from build123d import *

# Parameters (mm, degrees)
SKETCH2_W            = 12
SKETCH2_H            = 35.5
BOSS_EXTRUDE1_DEPTH  = 7.5
LPATTERN1_COUNT      = 2
LPATTERN1_PITCH      = 587
BOSS_EXTRUDE2_DEPTH  = 15
M5_CLEARANCE_HOLE1_D = 5.5
M5_CLEARANCE_HOLE2_D = 5.5


with BuildPart() as part:
    # Sketch1 → Revolve1 (revolve)
    with BuildSketch(Plane.XY):
        Polygon((0, 0), (0, 10.5), (29, 10.5), (29, 9.5), (39, 9.5), (39, 10.5), (75, 10.5), (75, 10), (625, 10), (625, 10.5), (661, 10.5), (661, 9.5), (671, 9.5), (671, 10.5), (700, 10.5), (700, 0), align=None)
    revolve(axis=Axis((700, 0, 0), (-1, 0, 0)))

    # Sketch2 → Boss-Extrude1 (add, symmetric)
    with BuildSketch(Plane.XY):
        with Locations((57, -7.25)):
            Rectangle(SKETCH2_W, SKETCH2_H)
    boss_extrude1 = extrude(amount=BOSS_EXTRUDE1_DEPTH, both=True)

    # LPattern1: Boss-Extrude1 ×2
    with Locations(*[(i * LPATTERN1_PITCH, 0, 0) for i in range(1, LPATTERN1_COUNT)]):
        add(boss_extrude1)

    # Sketch3 → Boss-Extrude2 (add)
    with BuildSketch(Plane(origin=(0, 10.5, 0), x_dir=(1, 0, 0), z_dir=(0, 1, 0))):
        Polygon((63, -7.5), (63, 0), (63, 7.5), (51, 7.5), (51, 0), (51, -7.5), align=None)
        Polygon((650, -7.5), (650, 0), (650, 7.5), (638, 7.5), (638, 0), (638, -7.5), align=None)
    extrude(amount=BOSS_EXTRUDE2_DEPTH)

    # M5 Clearance Hole1 (through all)
    with Locations(Plane(origin=(0, 25.5, 0), x_dir=(1, 0, 0), z_dir=(0, 1, 0))):
        with Locations((57, 0), (644, 0)):
            Hole(M5_CLEARANCE_HOLE1_D / 2)

    # M5 Clearance Hole2 (through all)
    with Locations(Plane.XY.offset(7.5)):
        with Locations((57, 17.5), (644, 17.5)):
            Hole(M5_CLEARANCE_HOLE2_D / 2)


solid = part.part
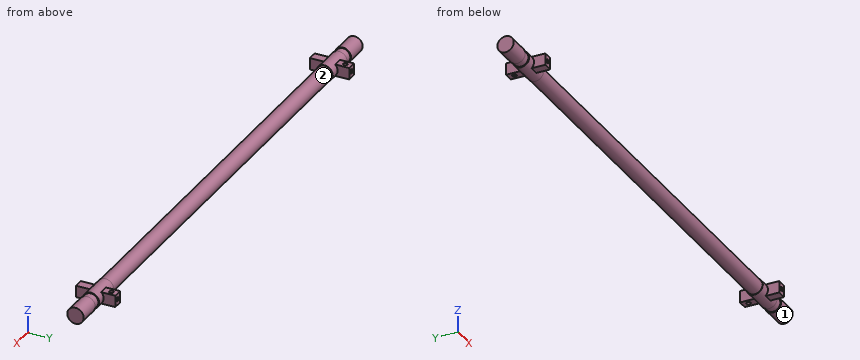
Could you check a few things on this model? Use its own coordinates, in mm. Face numbers are marked on the shaded views. A direction names the side the tool comes from. Give positions to 0.01 mm unless a question says otherwise; leave off trailing zeros. Order: outer loops, then holes, each group sorted by start corner. A loop starts at its lowest first (then second) coordinate and runs counter-clockwise, first axis right, second up. Notation, with made-up numbers: (78.25, 65.25) -> (120.25, 65.25) arc R17 cw to (120.25, 72.25) -> close; hole circle Ø2 at (65.25, 28). An arc over 180 degrees is marked (long way). Answer in a Markdown table with one row per item. Add a question column.
Item 1: I'm going to push flat-ended pins straight in: P1, Ø9, axis at x = 57, y = 17.5, coming from the -Z side; P2, Ø1, axis at x = 439.5, z = -5, coming from the -Y side; P3, Ø1, axis at x = 371, z = 6.5, coming from the +Y side; P4, Ø4.5, axis at x = 57, y = 17.5, coming from the +Z side. Where does each tip first touch, or does it pass through?
Item 2: For the marked faces 1 and 2, which set-ups out of +Z, -Z, +X, -X, +Y, -Y let a thin tool reach every point of the face, with its end or its side?
Item 3: Imagine slicing it at B-B (x = 83.5). List the corners of the cut face in (y, z) for me, and give its area (3 significant figures).
Item 4: Please list where these lines run through material, in increasing order: probe 1 along X at (y, z) = (18, 2.75); probe 2 along Y at (x, z) = (644, 4); probe 3 along X at (y, z) = (14, 5).
Item 5: Imagine slicing it at A-A (y = 0). Count the separate pieces of the cut face and the enclosed holes in it, and give its area (3 significant figures).
Result:
| question | item | result |
|---|---|---|
| 1 | P1 | z = -7.5 |
| 1 | P2 | y = -8.93 |
| 1 | P3 | y = 8 |
| 1 | P4 | through |
| 2 | face 1 | +X |
| 2 | face 2 | none |
| 3 | outline | circle Ø20 at (0, 0) |
| 3 | area | 314 mm2 |
| 4 | probe 1 | 51 to 54.3, 59.7 to 63, 638 to 641.3, 646.7 to 650 |
| 4 | probe 2 | -25 to 14.75, 20.25 to 25.5 |
| 4 | probe 3 | 51 to 63, 638 to 650 |
| 5 | separate pieces | 1 |
| 5 | enclosed holes | 2 |
| 5 | area | 14,100 mm2 |
